Part model, mm, in its own coordinate system. Face numbers are marked on the shaded views. A direction names the side the tool comes from. Round coordinates to 2 decimals unless told otherwise and drop trailing zeros. Order: outer loops, then holes, each group sorted by start corner. A loop starts at its lowest first (then second) coordinate and runs counter-clockwise, first axis right, second up. Notation, with made-up numbers: (-19.5, 31.5) -> (-8.5, 31.5) arc R32 cw to (-8.5, 58.5) -> close; hole circle Ø7 at (-27, -34). An arc over 180 degrees is marked (long way). Use CSV: the item, a comma, the result in double quotes.
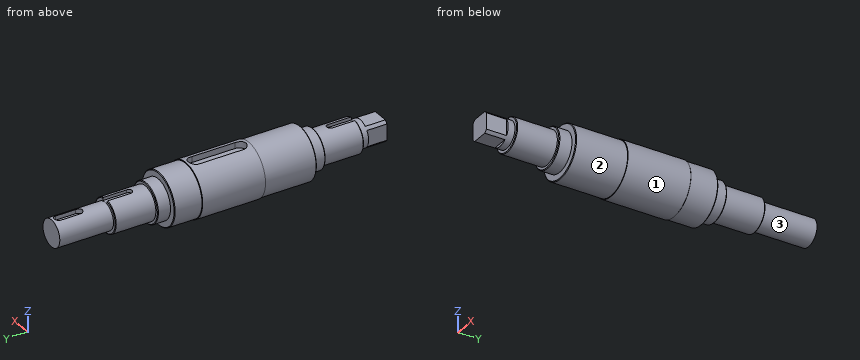
```python
from build123d import *

# Parameters (mm, degrees)
EXTRUDE1_DEPTH       = 32
EXTRUDE1_DEPTH_BACK  = 15
SKETCH1_R            = 20
SKETCH_1_R           = 19.5
EXTRUDE_1_DEPTH      = 38.5
EXTRUDE2_START       = 20.5
SKETCH2_R            = 19.5
EXTRUDE2_DEPTH       = 20.5
CHAMFER1_SIZE        = 0.2
CUT_EXTRUDE1_DEPTH   = 5
SKETCH5_R            = 14.75
EXTRUDE3_DEPTH       = 9.5
SKETCH6_R            = 12.5
EXTRUDE4_DEPTH       = 30
EXTRUDE5_START       = 9.5
SKETCH7_R            = 14.75
EXTRUDE5_DEPTH       = 9.5
EXTRUDE6_START       = 30
SKETCH8_R            = 12.5
EXTRUDE6_DEPTH       = 30
CHAMFER2_SIZE        = 0.5
SKETCH9_R            = 10
EXTRUDE7_DEPTH       = 40
CUT_EXTRUDE2_DEPTH   = 4.5
BOSS_EXTRUDE1_START  = 20
SKETCH11_R           = 10
BOSS_EXTRUDE1_DEPTH  = 20
SKETCH12_OUTSIDE_W   = 92.29
SKETCH12_OUTSIDE_H   = 92.29
SKETCH12_OUTSIDE_W_2 = 16
SKETCH12_OUTSIDE_H_2 = 16
CUT_EXTRUDE3_DEPTH   = 15
CHAMFER3_SIZE        = 0.5
CUT_EXTRUDE4_DEPTH   = 10


with BuildPart() as part:
    # Sketch1 → Extrude1 (new, two sides: drawn at the far end of the back side and taken through both)
    with BuildSketch(Plane(origin=(0, 0, 0), x_dir=(1, 0, 0), z_dir=(0, 1, 0)).offset(-EXTRUDE1_DEPTH_BACK)):
        with Locations(Location((0, 0, 0), (0, 0, 270))):
            Circle(SKETCH1_R)
    extrude(amount=EXTRUDE1_DEPTH + EXTRUDE1_DEPTH_BACK)

    # 草图1 → 拉伸1 (add)
    with BuildSketch(Plane.XZ.offset(15)):
        with Locations(Location((0, 0, 0), (0, 0, 90))):
            Circle(SKETCH_1_R)
    extrude(amount=EXTRUDE_1_DEPTH)

    # Sketch2 → Extrude2 (add)
    with BuildSketch(Plane(origin=(0, 32, 0), x_dir=(1, 0, 0), z_dir=(0, 1, 0)).offset(EXTRUDE2_START)):
        with Locations(Location((0, 0, 0), (0, 0, 270))):
            Circle(SKETCH2_R)
    extrude(amount=-EXTRUDE2_DEPTH)

    # Chamfer1
    chamfer1_edges = [part.edges().sort_by_distance(p)[0] for p in [
        (0, 32, -20),
    ]]
    chamfer(chamfer1_edges, length=CHAMFER1_SIZE)

    # Sketch4 → Cut-Extrude1 (cut)
    with BuildSketch(Plane.XY.offset(20)):
        with BuildLine():
            Line((-5, 26), (-5, -8))
            ThreePointArc((-5, -8), (0, -13), (5, -8))
            Line((5, -8), (5, 24))
            ThreePointArc((5, 24), (1, 30), (-5, 26))
        make_face()
    extrude(amount=-CUT_EXTRUDE1_DEPTH, mode=Mode.SUBTRACT)

    # Sketch5 → Extrude3 (add)
    with BuildSketch(Plane(origin=(0, 52.5, 0), x_dir=(1, 0, 0), z_dir=(0, 1, 0))):
        with Locations(Location((0, 0, 0), (0, 0, 270))):
            Circle(SKETCH5_R)
    extrude(amount=EXTRUDE3_DEPTH)

    # Sketch6 → Extrude4 (add)
    with BuildSketch(Plane(origin=(0, 62, 0), x_dir=(1, 0, 0), z_dir=(0, 1, 0))):
        with Locations(Location((0, 0, 0), (0, 0, 270))):
            Circle(SKETCH6_R)
    extrude(amount=EXTRUDE4_DEPTH)

    # Sketch7 → Extrude5 (add)
    with BuildSketch(Plane.XZ.offset(53.5).offset(EXTRUDE5_START)):
        with Locations(Location((0, 0, 0), (0, 0, 90))):
            Circle(SKETCH7_R)
    extrude(amount=-EXTRUDE5_DEPTH)

    # Sketch8 → Extrude6 (add)
    with BuildSketch(Plane.XZ.offset(63).offset(EXTRUDE6_START)):
        with Locations(Location((0, 0, 0), (0, 0, 90))):
            Circle(SKETCH8_R)
    extrude(amount=-EXTRUDE6_DEPTH)

    # Chamfer2
    chamfer2_edges = [part.edges().sort_by_distance(p)[0] for p in [
        (0, 52.5, -19.5),
        (0, 62, -14.75),
        (0, 92, -12.5),
        (0, -63, -14.75),
        (0, -53.5, -19.5),
    ]]
    chamfer(chamfer2_edges, length=CHAMFER2_SIZE)

    # Sketch9 → Extrude7 (add)
    with BuildSketch(Plane(origin=(0, 92, 0), x_dir=(1, 0, 0), z_dir=(0, 1, 0))):
        with Locations(Location((0, 0, 0), (0, 0, 270))):
            Circle(SKETCH9_R)
    extrude(amount=EXTRUDE7_DEPTH)

    # Sketch10 → Cut-Extrude2 (cut)
    with BuildSketch(Plane.XY.offset(11)):
        with BuildLine():
            Line((-3, 127), (-3, 112))
            ThreePointArc((-3, 112), (0, 109), (3, 112))
            Line((3, 112), (3, 127))
            ThreePointArc((3, 127), (0, 130), (-3, 127))
        make_face()
    extrude(amount=-CUT_EXTRUDE2_DEPTH, mode=Mode.SUBTRACT)

    # Sketch11 → Boss-Extrude1 (add)
    with BuildSketch(Plane.XZ.offset(93).offset(BOSS_EXTRUDE1_START)):
        with Locations(Location((0, 0, 0), (0, 0, 90))):
            Circle(SKETCH11_R)
    extrude(amount=-BOSS_EXTRUDE1_DEPTH)

    # Sketch12 outside → Cut-Extrude3 (cut)
    with BuildSketch(Plane.XZ.offset(113)):
        Rectangle(SKETCH12_OUTSIDE_W, SKETCH12_OUTSIDE_H)
        Rectangle(SKETCH12_OUTSIDE_W_2, SKETCH12_OUTSIDE_H_2, mode=Mode.SUBTRACT)
    extrude(amount=-CUT_EXTRUDE3_DEPTH, mode=Mode.SUBTRACT)

    # Chamfer3
    chamfer3_edges = [part.edges().sort_by_distance(p)[0] for p in [
        (0, -93, -12.5),
    ]]
    chamfer(chamfer3_edges, length=CHAMFER3_SIZE)

    # Sketch13 → Cut-Extrude4 (cut)
    with BuildSketch(Plane.XY.offset(10)):
        with BuildLine():
            Line((2.5, 92), (2.5, 74.5))
            ThreePointArc((2.5, 74.5), (0, 72), (-2.5, 74.5))
            Line((-2.5, 74.5), (-2.5, 92))
            ThreePointArc((-2.5, 92), (0, 94.5), (2.5, 92))
        make_face()
        with BuildLine():
            Line((-2.5, -93), (-2.5, -75.5))
            ThreePointArc((-2.5, -75.5), (0, -73), (2.5, -75.5))
            Line((2.5, -75.5), (2.5, -93))
            ThreePointArc((2.5, -93), (0, -95.5), (-2.5, -93))
        make_face()
    extrude(amount=CUT_EXTRUDE4_DEPTH, mode=Mode.SUBTRACT)


solid = part.part
```
(1) Drop flat-ended pins along their axis: P1, Ø6, axis at x = -7.5, y = -72.5, coming from the +Z side; P2, Ø5, axis at x = -9, y = -48, coming from the -Z side; P3, Ø1.5, axis at x = 9.5, y = 8, coming from the -Z side; P4, Ø12, axis at x = -8.5, z = 6, coming from the +Y side. Give the stop position or say it passes through.
Reply:
P1,"z = 11.66"
P2,"z = -18.38"
P3,"z = -17.98"
P4,"y = 132"
(2) Probe probe 1 along Z at (x, y) = (12.5, -48.5); probe 2 along Z at (x, y) = (1, -8.5); probe 3 along X at (y, z) = (29, 4.5). List the from-to ranges inside material, lowest first. Write a range as [from, to].
Reply:
probe 1,"[-14.97, 14.97]"
probe 2,"[-19.97, 15]"
probe 3,"[-19.49, 19.49]"
(3) Cut at A-A, the plane y = -69. Give the cut face in (x, z), then the cut area to 3 significant figures.
Reply:
outline,"circle Ø25 at (0, 0)"
area,"491 mm2"
(4) Which spindle directions (+Z, -Z, +X, -X, +Y, -Y) get a long thin tool onto all of the face, cutting with end or side? Do the marked faces 1, 2 and 3. Say none if no direction does.
Reply:
face 1,"+Y, -Y"
face 2,"-Y"
face 3,"+Y"
